Drawing for the job (mm, zero at the part's lowest x, y, z). A direction names the side the tool comes from. Round coordinates to 2 decimals unless told otherwise and drop trailing zeros. Order: outer loops, then holes, each group sorted by start corner. A loop starts at its lowest first (then second) coordinate and runs counter-clockwise, first axis right, second up. Notation, with made-up numbers: (44, 21.5) - (96, 21.5) arc R28 ccw to (96, 59.5) - close; hole circle Ø8 at (28.25, -12). An arc over 180 degrees is marked (long way). Answer as a JSON object with one key per item and string values.
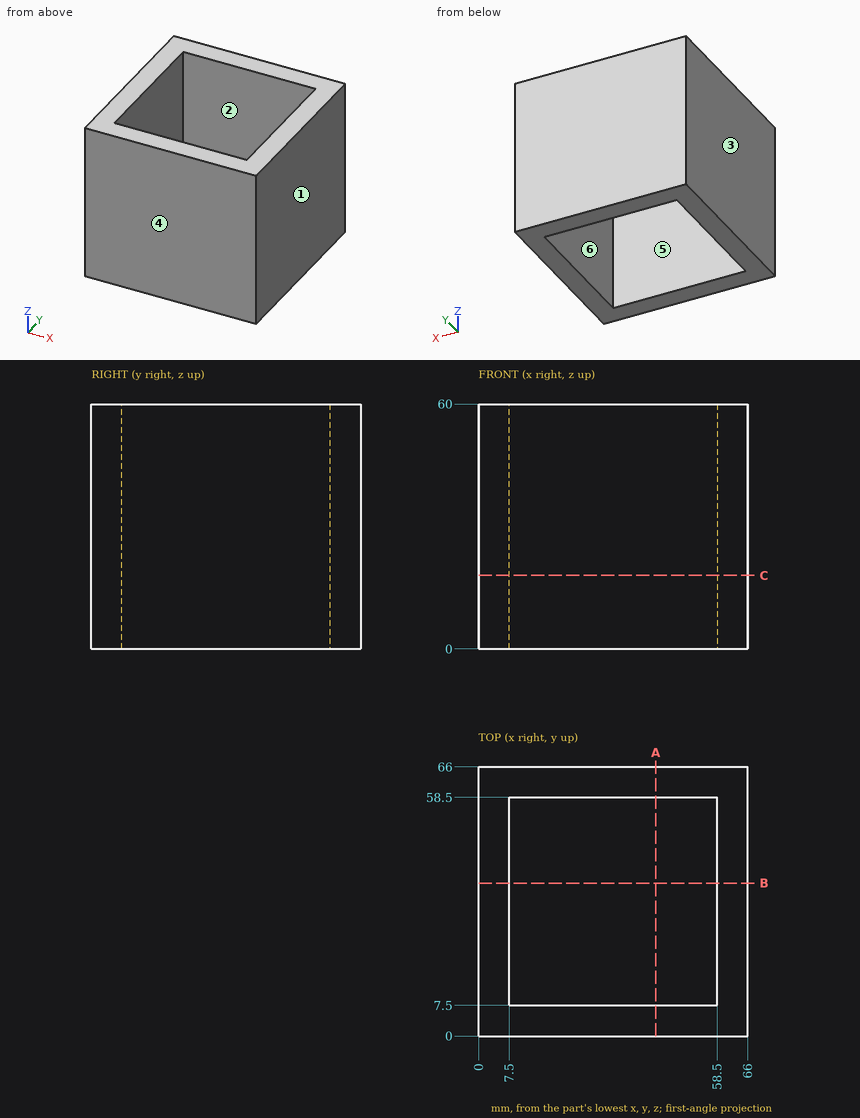
Item 1: Tool access for the marked faces 1 and 2: list every direction of +Z, -Z, +X, -X, +Y, -Y with a clear straight run to the whole face (end or side of a thin tool).
Taken from the geometry:
{"face 1": "+Z, -Z, +X, +Y, -Y", "face 2": "+Z, -Z"}
Item 2: Drop a flat-ended pin along its axis: P1, Ø6, axis at x = 20, y = 54.5, coming from the -Z side. Give the stop position or say it passes through.
Taken from the geometry:
{"P1": "through"}
Item 3: Cut at C-C (z = 18). Write the cut outline in (x, y).
Taken from the geometry:
{"outline": "(0, 0) - (66, 0) - (66, 66) - (0, 66) - close; hole (7.5, 7.5) - (58.5, 7.5) - (58.5, 58.5) - (7.5, 58.5) - close"}
Item 4: Probe L1, parallel to X at y = 29.5, z = 27. List the from-to ranges inside material, lowest first. Write a range as from..to.
Taken from the geometry:
{"L1": "0..7.5, 58.5..66"}
Item 5: Cut at A-A (x = 43.5). Write the cut outline in (y, z).
Taken from the geometry:
{"outline": "(0, 0) - (7.5, 0) - (7.5, 60) - (0, 60) - close; (58.5, 0) - (66, 0) - (66, 60) - (58.5, 60) - close"}
Item 6: Two-plate mould, pull along X, no slides. Class the marked faces 3, 4, 5 and 6: pulls with the +X half, pulls with the -X half, needs draft (parallel to the pull), parting line crosses it, or undercut.
Taken from the geometry:
{"face 3": "pulls with the -X half", "face 4": "needs draft", "face 5": "undercut", "face 6": "undercut"}
